Geometry: see drawing. Coordinates: mm, zero at the bounding-box minimum. Coordinates: 2 decimals unless noted, no trailing zeros. Write each loop counter-clockwise with the first axis right and the second up, starting at its lowest first coordinate (ties: lowest second). Pieces come first, ordered by that corner, then holes. Notation, with made-up numbers: M 22.25,16.5 L 57.25,16.5 A15 ccw 57.25,30.5 Z; hole C -3.5,49 d1. An arc over 180 degrees is marked long. Write item = value, one per line. Start each with the question number.
1. Section query A-A (y = 2.5). Output: boundary loops of the cut face in (x, z), then the cut area to 3 significant figures.
2. Line query: line 1 along Y through (x, z) = (14.5, 198); line 2 along Y through (x, z) = (25, 125). Output: solid intervals per line, ascending.
3. Pull-direction query (X, two-part tool) for the marked faces 1 and 2; classes: pulls with the +X half, pulls with the -X half, needs draft (parallel to the pull), parting line crosses it, or undercut.
4. Pin query (flat end, axial travel): pin 1 Ø12 at (x, z) = (15, 179) entering from -Y. Return the tip coordinate at first contact, or that it passes through.
5. Section query D-D (x = 7.5). Output: boundary loops of the cut face in (y, z).
6. Section query C-C (x = 24.5). Output: boundary loops of the cut face in (y, z), then the cut area to 3 significant figures.
7. Section query B-B (z = 185.5). Output: boundary loops of the cut face in (x, y).
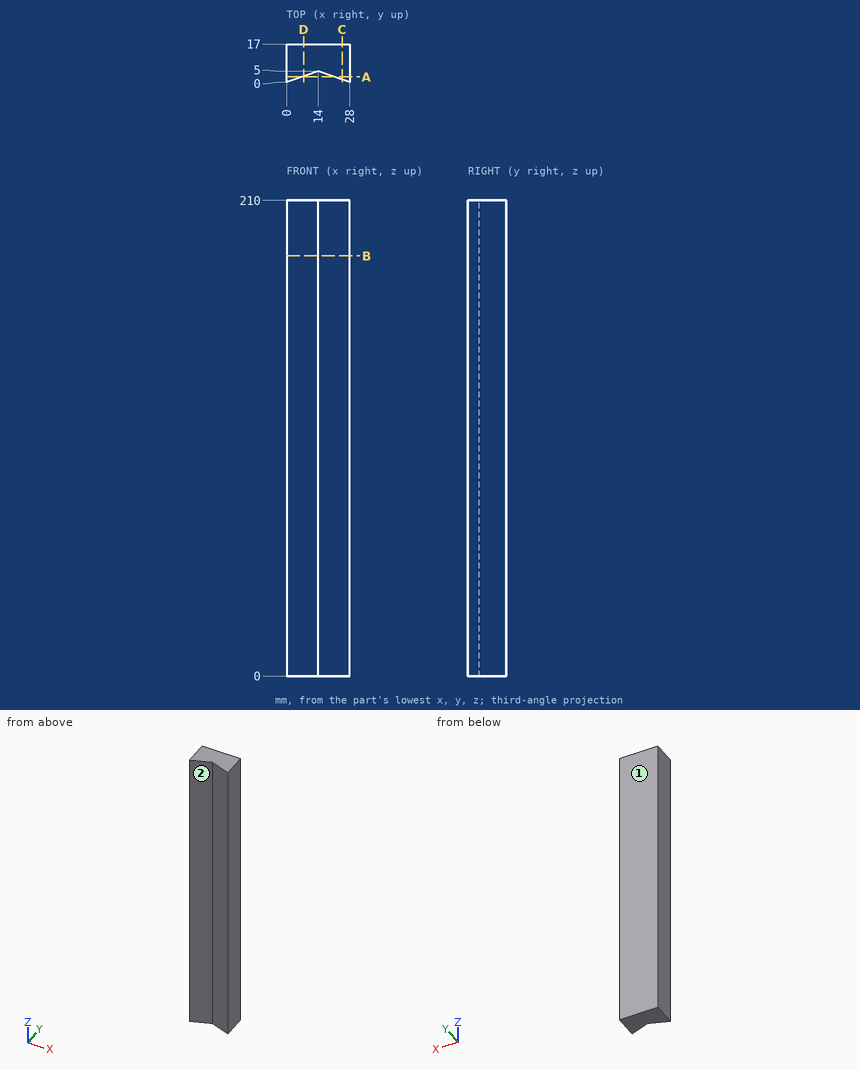
Results are:
q1.outline = M 0,0 L 7,0 L 7,210 L 0,210 Z; M 21,0 L 28,0 L 28,210 L 21,210 Z
q1.area = 2,940 mm^2
q2.line_1 = 4.82 to 17
q2.line_2 = 1.07 to 17
q3.face_1 = needs draft
q3.face_2 = undercut
q4.pin_1 = 2.5
q5.outline = M 2.68,0 L 17,0 L 17,210 L 2.68,210 Z
q6.outline = M 1.25,0 L 17,0 L 17,210 L 1.25,210 Z
q6.area = 3,310 mm^2
q7.outline = M 0,0 L 14,5 L 28,0 L 28,17 L 0,17 Z
